Source: CAD feature listing. Evaluate the final solid. Frame: model axes, mm. A direction names the side the tool comes from. Coordinates: 2 decimals unless noted, no trailing zeros. Order: outer loops, then holes, each group sorted by start corner. A loop starts at its lowest first (then second) coordinate and runs counter-clockwise, first axis right, second up. Notation, with made-up numbers: (51.25, -15.5) -> (55.25, -15.5) arc R7 ccw to (55.25, -6.5) -> close; hole circle Ø6 at (89.25, 53.5). An arc over 180 degrees is marked (long way). Write item = value, one per line. Start each with the question number.
Item 1: Section query A-A (x = 0). Output: boundary loops of the cut face in (y, z), then the cut area to 3 significant figures.
Item 2: Mould query, pull axis Y, two halves, no side actions, for faces 4 (the cylindrical face through (-77, 0, 16)), 5 (the cylindrical face through (-39.747, -50.303, 7.888)), 6 (the cylindrical face through (154, 0, 30)), 7 (the flat face through (-12.99, 54.5, 7.89)). Classes: released by +Y, released by -Y, zero draft, split by the parting line, or undercut.
Item 3: Ray query, line 1 along X through (y, z) = (-4, 16); line 2 along Y through (x, z) = (62.5, 37.5); line 3 along Y through (x, z) = (70, 20.5). Return the intervals inside material, ascending. Write a range as [from, to].
Item 4: Section query C-C (x = 75). Output: boundary loops of the cut face in (y, z), then the cut area to 3 significant figures.
Item 5: Contact query for flat-ended pins moving along their axis: pin 1 (1.5 mm diameter, centred on y = 9.5, z = 27, fed in from +X); pin 2 (16 mm diameter, centred on x = -32.5, y = 56.29, fed in from -Z); pin 3 (6 mm diameter, centred on x = 51.5, y = 2, fed in from -Z); pin 4 (2 mm diameter, centred on y = 38.5, z = 54, fed in from -X). Output: stop coordinate, or through.
Item 6: Section query B-B (z = 26.5). Output: boundary loops of the cut face in (x, y), then the cut area to 3 significant figures.
Item 7: Set-up query: faces 1 (the flat face through (-40.54, 38.22, 7.89)), 2 (the flat face through (-30, -49, 16)), 3 (the flat face through (91.036, -14.233, 29.79)). Return all of +Z, -Z, +X, -X, +Y, -Y with unobstructed straight access to the full face (end or side cutting, diameter ignored); none if empty.
Item 8: Section query D-D (z = 52). Output: boundary loops of the cut face in (x, y), then the cut area to 3 significant figures.
```python
from build123d import *

# Parameters (mm, degrees)
HUB_PROFILE_90X_64_R   = 45
HUB_PROFILE_90X_64_R_2 = 32
HUB_90X_64_DEPTH       = 60
ARM_WEB_PROFILE_R      = 6
WEBBED_ARM_DEPTH       = 15
LUG_A_PROFILE_R        = 7
LUG_A_30DEG_DEPTH      = 16
LUG_B_PROFILE_R        = 7
LUG_B_30DEG_DEPTH      = 16
LUG_BOSS_DEPTH         = 8
LUG_HOLE_PROFILE_R     = 7
LUG_THROUGH_HOLE_DEPTH = 16


with BuildPart() as part:
    # Hub Profile Ø90xØ64 → Hub Ø90xØ64 (new body)
    with BuildSketch(Plane.XY):
        Circle(HUB_PROFILE_90X_64_R)
        Circle(HUB_PROFILE_90X_64_R_2, mode=Mode.SUBTRACT)
    extrude(amount=HUB_90X_64_DEPTH)

    # Arm Web Profile → Webbed Arm (add, symmetric)
    with BuildSketch(Plane.XY.offset(30)):
        with BuildLine():
            Line((10.457746479, -43.767973892), (144.788732394, -11.671459704))
            ThreePointArc((144.788732394, -11.671459704), (154, 0), (144.788732394, 11.671459704))
            Line((144.788732394, 11.671459704), (10.457746479, 43.767973892))
            ThreePointArc((10.457746479, 43.767973892), (45, 0), (10.457746479, -43.767973892))
        make_face()
        with Locations((142, 0)):
            Circle(ARM_WEB_PROFILE_R, mode=Mode.SUBTRACT)
        with BuildLine():
            ThreePointArc((127.907920927, -5.423403672), (129.71316959, -4.160179273), (130.168590262, -2.004430997))
            ThreePointArc((130.168590262, -2.004430997), (130, 0), (130.168590262, 2.004430997))
            ThreePointArc((130.168590262, 2.004430997), (129.71316959, 4.160179273), (127.907920927, 5.423403672))
            Line((127.907920927, 5.423403672), (49.398644334, 24.182099536))
            ThreePointArc((49.398644334, 24.182099536), (54.923721956, 2.89564613), (51.667548043, -18.853765651))
            ThreePointArc((51.667548043, -18.853765651), (52.245702855, -21.877663737), (55.182961035, -22.800017794))
            Line((55.182961035, -22.800017794), (127.907920927, -5.423403672))
        make_face(mode=Mode.SUBTRACT)
    extrude(amount=WEBBED_ARM_DEPTH, both=True)

    # Lug A Profile → Lug A 30deg (add)
    with BuildSketch(Plane.XY):
        with BuildLine():
            Line((-34.886147305, 28.424579613), (-46.356406461, 48.291651246))
            ThreePointArc((-46.356406461, 48.291651246), (-40.5, 70.148057707), (-18.643593539, 64.291651246))
            Line((-18.643593539, 64.291651246), (-7.173334384, 44.424579613))
            ThreePointArc((-7.173334384, 44.424579613), (-22.5, 38.97114317), (-34.886147305, 28.424579613))
        make_face()
        with Locations((-32.5, 56.291651246)):
            Circle(LUG_A_PROFILE_R, mode=Mode.SUBTRACT)
    extrude(amount=LUG_A_30DEG_DEPTH)

    # Lug B Profile → Lug B 30deg (add)
    with BuildSketch(Plane.XY):
        with BuildLine():
            ThreePointArc((-8.833624625, -44.124449866), (-23.945086023, -38.100299938), (-35.927171248, -27.096833139))
            Line((-35.927171248, -27.096833139), (-48.134119789, -46.519958213))
            ThreePointArc((-48.134119789, -46.519958213), (-43.101154841, -68.580539888), (-21.040573166, -63.547574941))
            Line((-21.040573166, -63.547574941), (-8.833624625, -44.124449866))
        make_face()
        with Locations((-34.587346477, -55.033766577)):
            Circle(LUG_B_PROFILE_R, mode=Mode.SUBTRACT)
    extrude(amount=LUG_B_30DEG_DEPTH)

    # Lug Boss Profile → Lug Boss (add, symmetric)
    with BuildSketch(Plane(origin=(0, 0, 0), x_dir=(1, 0, 0), z_dir=(0, 1, 0))):
        with BuildLine():
            Line((-61, 0), (-45, 0))
            Line((-45, 0), (-39.05307602, 0))
            Line((-39.05307602, 0), (-39.05307602, -32))
            Line((-39.05307602, -32), (-45, -32))
            Line((-45, -32), (-61, -32))
            ThreePointArc((-61, -32), (-77, -16), (-61, 0))
        make_face()
    extrude(amount=LUG_BOSS_DEPTH, both=True)

    # Lug Hole Profile → Lug Through Hole (cut)
    with BuildSketch(Plane(origin=(0, 8, 0), x_dir=(1, 0, 0), z_dir=(0, 1, 0))):
        with Locations(Location((-61, -16, 0), (0, 0, 270))):
            Circle(LUG_HOLE_PROFILE_R)
    extrude(amount=-LUG_THROUGH_HOLE_DEPTH, mode=Mode.SUBTRACT)


solid = part.part
```
Computed:
q1.outline = (-45, 0) -> (-32, 0) -> (-32, 60) -> (-45, 60) -> close; (32, 0) -> (45, 0) -> (45, 60) -> (32, 60) -> close
q1.area = 1,560 mm^2
q2.face_4 = zero draft
q2.face_5 = undercut
q2.face_6 = split by the parting line
q2.face_7 = released by +Y
q3.line_1 = [-77, -68], [-54, -31.75], [31.75, 54.85], [129.81, 137.53], [146.47, 153.31]
q3.line_2 = [-31.33, -21.05], [21.05, 31.33]
q3.line_3 = [-29.54, -19.26], [19.26, 29.54]
q4.outline = (-28.35, 15) -> (-18.07, 15) -> (-18.07, 45) -> (-28.35, 45) -> close; (18.07, 15) -> (28.35, 15) -> (28.35, 45) -> (18.07, 45) -> close
q4.area = 617 mm^2
q5.pin_1 = 150.21
q5.pin_2 = 0
q5.pin_3 = 15
q5.pin_4 = -24.87
q6.outline = (-73.07, -8) -> (-44.28, -8) arc R45 ccw to (10.46, -43.77) -> (144.79, -11.67) arc R12 ccw to (144.79, 11.67) -> (10.46, 43.77) arc R45 ccw to (-44.28, 8) -> (-73.07, 8) -> close; hole circle Ø64 at (0, 0); hole (49.4, 24.18) arc R55 cw to (51.67, -18.85) arc R3 ccw to (55.18, -22.8) -> (127.91, -5.42) arc R3 ccw to (130.17, -2) arc R12 cw to (130.17, 2) arc R3 ccw to (127.91, 5.42) -> close; hole circle Ø12 at (142, 0)
q6.area = 6,690 mm^2
q7.face_1 = +Z, -Z, -X
q7.face_2 = +Z, -X, -Y
q7.face_3 = +Z, -Z
q8.outline = circle Ø90 at (0, 0); hole circle Ø64 at (0, 0)
q8.area = 3,140 mm^2
